Model file for the job. Use its own axes, mm. Coordinates: 2 decimals unless noted, no trailing zeros. Write each loop counter-clockwise with the first axis right and the second up, starting at its lowest first coordinate (ties: lowest second). Pieces come first, ordered by that corner, then holes. Notation, with made-up numbers: M -38.5,89 L -34.5,89 A25 ccw -34.5,113 Z; hole C 73.25,21.25 d2. An arc over 180 degrees is marked long. One line per question, with ' | ' between items. Start each with the question number.
(1) Cut at B-B (x = 8.25). Write the cut outline in (y, z), plus the area to 3 significant figures.
(2) Cut at A-A (y = -3.5). Write the cut outline in (x, z), plus the area to 3 significant figures.
(3) Cut at C-C (z = -0.55). Write the cut outline in (x, y), plus the area to 3 significant figures.
(4) Flat gauge pin, fed straight in: pin 1 Ø2.5 at (x, y) = (-5.09, -7.06) entering from -Z. Where does the tip first touch, or does it go through?
(5) Wall check: probe 1 along X at (y, z) = (-7.5, -0.75); probe 2 along Y at (x, z) = (-3.75, -0.45); probe 3 along Y at (x, z) = (-8, -0.1). Give the ranges that are in metal, low to high.
(6) Cut at D-D (x = 0). Write the cut outline in (y, z).
from build123d import *

# Parameters (mm, degrees)
SKETCH1_R  = 1
BODY_DEPTH = 1


with BuildPart() as part:
    # Sketch1 → Body (new body)
    with BuildSketch(Plane.XY):
        with BuildLine():
            Line((-2.410905624, -5.820441055), (-4.113846898, -9.931704974))
            ThreePointArc((-4.113846898, -9.931704974), (0, 10.75), (4.113846898, -9.931704974))
            Line((4.113846898, -9.931704974), (2.410905624, -5.820441055))
            ThreePointArc((2.410905624, -5.820441055), (4.232413877, -4.666548272), (5.558129248, -2.966007293))
            ThreePointArc((5.558129248, -2.966007293), (7.908430264, -2.290246226), (8.83133721, -0.025558466))
            ThreePointArc((8.83133721, -0.025558466), (0, 8.25), (-8.83133721, -0.025558466))
            ThreePointArc((-8.83133721, -0.025558466), (-7.908430264, -2.290246226), (-5.558129248, -2.966007293))
            ThreePointArc((-5.558129248, -2.966007293), (-4.232413877, -4.666548272), (-2.410905624, -5.820441055))
        make_face()
        with Locations(Location((5.087937676, -7.057116281, 0), (0, 0, 180))):
            Circle(SKETCH1_R, mode=Mode.SUBTRACT)
        with Locations((-5.087937676, -7.057116281)):
            Circle(SKETCH1_R, mode=Mode.SUBTRACT)
    extrude(amount=-BODY_DEPTH)


solid = part.part
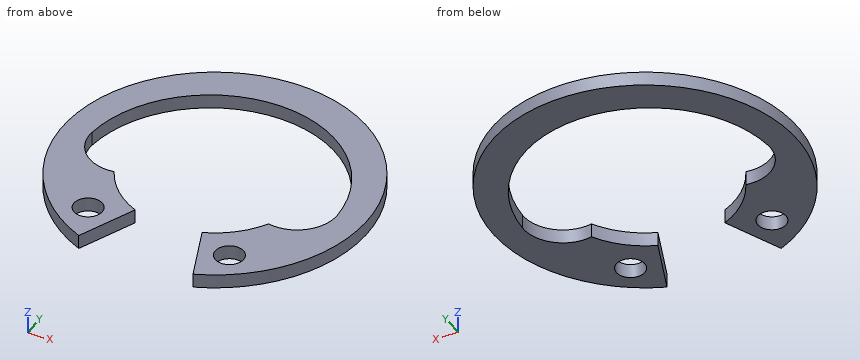
Filled in:
1) outline: M -6.89,-1 L -1.92,-1 L -1.92,0 L -6.89,0 Z; M 2.6,-1 L 6.89,-1 L 6.89,0 L 2.6,0 Z | area: 9.26 mm²
2) outline: M -10.16,-1 L -5.24,-1 L -5.24,0 L -10.16,0 Z; M 5.24,-1 L 10.16,-1 L 10.16,0 L 5.24,0 Z | area: 9.85 mm²
3) outline: M -8.83,-0.03 A8.85 cw 8.83,-0.03 A2.8 cw 5.56,-2.97 A6.3 cw 2.41,-5.82 L 4.11,-9.93 A10.75 ccw long -4.11,-9.93 L -2.41,-5.82 A6.3 cw -5.56,-2.97 A2.8 cw Z; hole C -5.09,-7.06 d2; hole C 5.09,-7.06 d2 | area: 139 mm²
4) pin 1: z = -1
5) probe 1: -7.7 to -5.98, -4.19 to -3.11, 3.11 to 4.19, 5.98 to 7.7 | probe 2: -9.05 to -5.06, 7.42 to 10.07 | probe 3: -7.18 to -2.2, 3.18 to 7.18
6) outline: M 8.25,-1 L 10.75,-1 L 10.75,0 L 8.25,0 Z
